```python
from build123d import *

# Parameters (mm, degrees)
SKETCH_1_R      = 31.5
SKETCH_1_R_2    = 25
EXTRUDE_1_DEPTH = 23.5
CHAMFER_1_SIZE  = 0.5


with BuildPart() as part:
    # 草图1 → 凸台-拉伸1 (new body)
    with BuildSketch(Plane.XY):
        Circle(SKETCH_1_R)
        Circle(SKETCH_1_R_2, mode=Mode.SUBTRACT)
    extrude(amount=EXTRUDE_1_DEPTH)

    # 倒角1
    chamfer_1_edges = [part.edges().sort_by_distance(p)[0] for p in [
        (-31.5, 0, 0),
        (-31.5, 0, 23.5),
        (-25, 0, 0),
        (-25, 0, 23.5),
    ]]
    chamfer(chamfer_1_edges, length=CHAMFER_1_SIZE)


solid = part.part
```
Build history of the part. All positions in model axes, mm. Round coordinates to 2 decimals unless told otherwise and drop trailing zeros. Loops run counter-clockwise (first coordinate to the right, second up) from the corner with the lowest first, then second, coordinate; pieces in that order, holes last. Notation, with made-up numbers: M -8,66.5 L 16,66.5 A10 cw 16,79.5 Z; hole C 68.5,8 d11. An arc over 180 degrees is marked long. Answer as CSV lines item,"result".
1. Cut at C-C on z = 6.5. Write the cut outline in (x, y).
Resolved:
outline,"C 0,0 d63; hole C 0,0 d50"
2. Wall check: probe 1 along Y at (x, z) = (0, 8.5); probe 2 along X at (y, z) = (8.5, 20.75); probe 3 along X at (y, z) = (-1.5, 21.25). Give the ranges that are in metal, low to high. Write a range as [from, to].
Resolved:
probe 1,"y = [-31.5, -25], [25, 31.5]"
probe 2,"x = [-30.33, -23.51], [23.51, 30.33]"
probe 3,"x = [-31.46, -24.95], [24.95, 31.46]"
3. Cut at A-A on y = 0. Write the cut outline in (x, z), then the cut area to 4 significant figures.
Resolved:
outline,"M -31.5,0.5 L -31,0 L -25.5,0 L -25,0.5 L -25,23 L -25.5,23.5 L -31,23.5 L -31.5,23 Z; M 25,0.5 L 25.5,0 L 31,0 L 31.5,0.5 L 31.5,23 L 31,23.5 L 25.5,23.5 L 25,23 Z"
area,"304.5 mm²"
4. Flat gauge pins, fed straight in: P1, Ø1.5, axis at y = 22.5, z = 2.5, coming from the +X side; P2, Ø12, axis at y = 14, z = 6, coming from the +X side; P3, Ø1.5, axis at y = -19.5, z = 11.5, coming from the -X side; P4, Ø6, axis at x = -23.5, y = 15.5, coming from the -Z side. Where does each tip first touch, or does it go through?
Resolved:
P1,"stops at x = 22.79"
P2,"stops at x = 30.47"
P3,"stops at x = -25.31"
P4,"stops at z = 0"
5. Two-plate mould, pull along X, no slides. Class faces 1 (the cylindrical face through (-4.101, 31.232, 11.592)), 2 (the flat face through (-12, -23, 23.5)), 3 (the cylindrical face through (23.846, 7.509, 11.592)): released by +X, released by -X, zero draft, split by the parting line, or undercut.
Resolved:
face 1,"split by the parting line"
face 2,"zero draft"
face 3,"undercut"
